Could you check a few things on this model? Use its own coordinates, in mm. A direction names the side the tool comes from. Coordinates: 2 decimals unless noted, no trailing zeros. Loops run counter-clockwise (first coordinate to the right, second up) from the corner with the lowest first, then second, coordinate; pieces in that order, holes last.
1) If I drill on line 1 along Y through (x, z) = (95, 4.25); line 2 along Y through (x, z) = (-25, 10.5); line 3 along X through (y, z) = (36, 11.25), over which ranges is the centre line in solid material (lowest first)?
2) For faces 4 (the face through (-98.37, -57.59, 6.41)), 5 (the face through (-113, 44, 11)), which set-ups out of +Z, -Z, +X, -X, +Y, -Y let a thin tool reach every point of the face, with its end or its side?
3) Imagine slicing it at C-C on z = 5.5. Give the number of separate pieces and of enclosed holes in the cut face, plus the area to 3 significant figures.
4) Imagine slicing it at A-A on y = -55. Please give me the cut outline in (x, z).
5) Imagine slicing it at D-D on y = 8.5. Please give me the cut outline in (x, z), plus the area to 3 significant figures.
6) Thinking about a two-plate mould opening in Y: for faces 1 (the face through (-135, 1, 8)), 2 (the face through (91.63, -57.59, 6.41)), 3 (the face through (2, 65, 8)), which applies, released by +Y, released by -Y, zero draft, split by the parting line, or undercut?
7) Imagine slicing it at B-B on x = 125. Please give me the cut outline in (y, z).
```python
from build123d import *

# Parameters (mm, degrees)
SKETCH_1_R      = 4.25
EXTRUDE_1_DEPTH = 10
SKETCH_2_R      = 4.25
EXTRUDE_2_DEPTH = 3
FILLET_1_R      = 3


with BuildPart() as part:
    # 草图1 → 凸台-拉伸1 (new body)
    with BuildSketch(Plane.XY):
        with BuildLine():
            Line((-132, -65), (132, -65))
            ThreePointArc((132, -65), (134.121320344, -64.121320344), (135, -62))
            Line((135, -62), (135, 62))
            ThreePointArc((135, 62), (134.121320344, 64.121320344), (132, 65))
            Line((132, 65), (-132, 65))
            ThreePointArc((-132, 65), (-134.121320344, 64.121320344), (-135, 62))
            Line((-135, 62), (-135, -62))
            ThreePointArc((-135, -62), (-134.121320344, -64.121320344), (-132, -65))
        make_face()
        with Locations((-125, 55)):
            Circle(SKETCH_1_R, mode=Mode.SUBTRACT)
        with Locations((-95, 55)):
            Circle(SKETCH_1_R, mode=Mode.SUBTRACT)
        with Locations((0, 55)):
            Circle(SKETCH_1_R, mode=Mode.SUBTRACT)
        with Locations((95, 55)):
            Circle(SKETCH_1_R, mode=Mode.SUBTRACT)
        with Locations((125, 55)):
            Circle(SKETCH_1_R, mode=Mode.SUBTRACT)
        with Locations((125, -55)):
            Circle(SKETCH_1_R, mode=Mode.SUBTRACT)
        with Locations((95, -55)):
            Circle(SKETCH_1_R, mode=Mode.SUBTRACT)
        with Locations((0, -55)):
            Circle(SKETCH_1_R, mode=Mode.SUBTRACT)
        with Locations((-95, -55)):
            Circle(SKETCH_1_R, mode=Mode.SUBTRACT)
        with Locations((-125, -55)):
            Circle(SKETCH_1_R, mode=Mode.SUBTRACT)
    extrude(amount=EXTRUDE_1_DEPTH)

    # 草图2 → 凸台-拉伸2 (add)
    with BuildSketch(Plane.XY.offset(10)):
        with BuildLine():
            Line((132, 65), (-132, 65))
            ThreePointArc((-132, 65), (-134.121320344, 64.121320344), (-135, 62))
            Line((-135, 62), (-135, -62))
            ThreePointArc((-135, -62), (-134.121320344, -64.121320344), (-132, -65))
            Line((-132, -65), (132, -65))
            ThreePointArc((132, -65), (134.121320344, -64.121320344), (135, -62))
            Line((135, -62), (135, 62))
            ThreePointArc((135, 62), (134.121320344, 64.121320344), (132, 65))
        make_face()
        with Locations((-125, -55)):
            Circle(SKETCH_2_R, mode=Mode.SUBTRACT)
        with Locations((-95, -55)):
            Circle(SKETCH_2_R, mode=Mode.SUBTRACT)
        with Locations((0, -55)):
            Circle(SKETCH_2_R, mode=Mode.SUBTRACT)
        with Locations((95, -55)):
            Circle(SKETCH_2_R, mode=Mode.SUBTRACT)
        with Locations((125, -55)):
            Circle(SKETCH_2_R, mode=Mode.SUBTRACT)
        with Locations((125, 55)):
            Circle(SKETCH_2_R, mode=Mode.SUBTRACT)
        with Locations((95, 55)):
            Circle(SKETCH_2_R, mode=Mode.SUBTRACT)
        with Locations((0, 55)):
            Circle(SKETCH_2_R, mode=Mode.SUBTRACT)
        with Locations((-95, 55)):
            Circle(SKETCH_2_R, mode=Mode.SUBTRACT)
        with Locations((-125, 55)):
            Circle(SKETCH_2_R, mode=Mode.SUBTRACT)
        with BuildLine():
            Line((-110, -45), (110, -45))
            ThreePointArc((110, -45), (113.535533906, -43.535533906), (115, -40))
            Line((115, -40), (115, 40))
            ThreePointArc((115, 40), (113.535533906, 43.535533906), (110, 45))
            Line((110, 45), (-110, 45))
            ThreePointArc((-110, 45), (-113.535533906, 43.535533906), (-115, 40))
            Line((-115, 40), (-115, -40))
            ThreePointArc((-115, -40), (-113.535533906, -43.535533906), (-110, -45))
        make_face(mode=Mode.SUBTRACT)
    extrude(amount=EXTRUDE_2_DEPTH)

    # 圆角1
    fillet_1_edges = [part.edges().sort_by_distance(p)[0] for p in [
        (0, 65, 0),
        (134.121320344, 64.121320344, 0),
        (135, 0, 0),
        (134.121320344, -64.121320344, 0),
        (0, -65, 0),
        (-134.121320344, -64.121320344, 0),
        (-135, 0, 0),
        (-134.121320344, 64.121320344, 0),
    ]]
    fillet(fillet_1_edges, radius=FILLET_1_R)


solid = part.part
```
Filled in:
1. line 1: y = -65 to -59.25, -50.75 to 50.75, 59.25 to 65
1. line 2: y = -65 to -45, 45 to 65
1. line 3: x = -135 to -115, 115 to 135
2. face 4: +Z, -Z
2. face 5: +Z
3. separate pieces: 1
3. enclosed holes: 10
3. area: 34,500 mm2
4. outline: (-135, 3) arc R3 ccw to (-132, 0) - (-129.25, 0) - (-129.25, 13) - (-135, 13) - close; (-120.75, 0) - (-99.25, 0) - (-99.25, 13) - (-120.75, 13) - close; (-90.75, 0) - (-4.25, 0) - (-4.25, 13) - (-90.75, 13) - close; (4.25, 0) - (90.75, 0) - (90.75, 13) - (4.25, 13) - close; (99.25, 0) - (120.75, 0) - (120.75, 13) - (99.25, 13) - close; (129.25, 0) - (132, 0) arc R3 ccw to (135, 3) - (135, 13) - (129.25, 13) - close
5. outline: (-135, 3) arc R3 ccw to (-132, 0) - (132, 0) arc R3 ccw to (135, 3) - (135, 13) - (115, 13) - (115, 10) - (-115, 10) - (-115, 13) - (-135, 13) - close
5. area: 2,820 mm2
6. face 1: zero draft
6. face 2: undercut
6. face 3: released by +Y
7. outline: (-65, 3) arc R3 ccw to (-62, 0) - (-59.25, 0) - (-59.25, 13) - (-65, 13) - close; (-50.75, 0) - (50.75, 0) - (50.75, 13) - (-50.75, 13) - close; (59.25, 0) - (62, 0) arc R3 ccw to (65, 3) - (65, 13) - (59.25, 13) - close
